from build123d import *

# Parameters (mm, degrees)
BOSS_EXTRUDE1_DEPTH      = 600
SKETCH2_R                = 15
BOSS_EXTRUDE2_DEPTH      = 30
BOSS_EXTRUDE3_DEPTH      = 12
BOSS_EXTRUDE3_DEPTH_BACK = 12
SKETCH3_R                = 15
SKETCH4_W                = 64.999273694
SKETCH4_H                = 54.968001075
CUT_EXTRUDE1_DEPTH       = 5
CUT_EXTRUDE2_DEPTH       = 621.826062597


with BuildPart() as part:
    # Sketch1 → Boss-Extrude1 (new body)
    with BuildSketch(Plane(origin=(0, 0, 0), x_dir=(1, 0, 0), z_dir=(0, 1, 0))):
        Polygon((-20, 40), (-20, 60), (50, 60), (50, -60), (-20, -60), (-20, -40), (20, -40), (20, 40), align=None)
    extrude(amount=BOSS_EXTRUDE1_DEPTH)

    # Sketch2 → Boss-Extrude2 (add)
    with BuildSketch(Plane(origin=(0, 0, -60), x_dir=(-1, 0, 0), z_dir=(0, 0, -1))):
        with BuildLine():
            Line((-34.984231122, 36.653571932), (-80, 36.653571932))
            ThreePointArc((-80, 36.653571932), (-105, 61.653571932), (-80, 86.653571932))
            Line((-80, 86.653571932), (-34.984231122, 86.653571932))
            Line((-34.984231122, 86.653571932), (-34.984231122, 36.653571932))
        make_face()
        with Locations((-80, 61.653571932)):
            Circle(SKETCH2_R, mode=Mode.SUBTRACT)
    boss_extrude2 = extrude(amount=-BOSS_EXTRUDE2_DEPTH)

    # Mirror1: Boss-Extrude2 across plane
    add(boss_extrude2.mirror(Plane.XY))

    # Sketch3 → Boss-Extrude3 (add, two sides: drawn at the far end of the back side and taken through both)
    with BuildSketch(Plane.XY.offset(-BOSS_EXTRUDE3_DEPTH_BACK)):
        with BuildLine():
            Line((42.373646318, 600), (75, 600))
            ThreePointArc((75, 600), (100, 575), (75, 550))
            Line((75, 550), (42.373646318, 550))
            Line((42.373646318, 550), (42.373646318, 600))
        make_face()
        with Locations((75, 575)):
            Circle(SKETCH3_R, mode=Mode.SUBTRACT)
    extrude(amount=BOSS_EXTRUDE3_DEPTH + BOSS_EXTRUDE3_DEPTH_BACK)

    # Sketch4 → Cut-Extrude1 (cut)
    with BuildSketch(Plane(origin=(0, 0, -60), x_dir=(-1, 0, 0), z_dir=(0, 0, -1))):
        with Locations((-82.499636847, 64.13757247)):
            Rectangle(SKETCH4_W, SKETCH4_H)
    cut_extrude1 = extrude(amount=-CUT_EXTRUDE1_DEPTH, mode=Mode.SUBTRACT)

    # Mirror2: Cut-Extrude1 across plane
    add(cut_extrude1.mirror(Plane.XY), mode=Mode.SUBTRACT)

    # Sketch5 → Cut-Extrude2 (cut, through all)
    with BuildSketch(Plane(origin=(0, 0, -60), x_dir=(-1, 0, 0), z_dir=(0, 0, -1))):
        Polygon((-50, 30.340627067), (-30, 0), (-50, 0), align=None)
    extrude(amount=-CUT_EXTRUDE2_DEPTH, mode=Mode.SUBTRACT)


solid = part.part
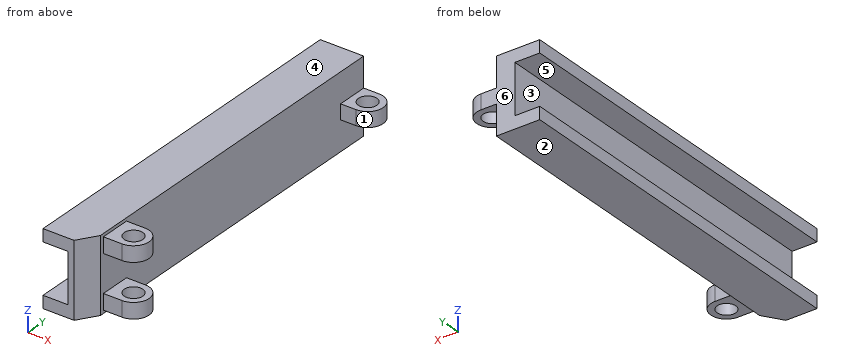
Input: part model. Units: mm. Frame: model coordinates. Face numbers are marked on the shaded views. A direction names the side the tool comes from. Give positions to 0.01 mm unless a question says otherwise; leave off trailing zeros. Loops run counter-clockwise (first coordinate to the right, second up) from the corner with the lowest first, then second, coordinate; pieces in that order, holes last. Notation, with made-up numbers: M 41,53.5 L 47,53.5 A16 cw 47,62.5 Z; hole C -11,60 d5. An arc over 180 degrees is marked long. Use CSV: the item, a comma, the result in double quotes.
(1) Section A-A, the plane y = 575. Return loops of the section in (x, z).
Outcome:
outline,"M -20,-60 L 50,-60 L 50,-12 L 60,-12 L 60,12 L 50,12 L 50,60 L -20,60 L -20,40 L 20,40 L 20,-40 L -20,-40 Z; M 90,-12 L 100,-12 L 100,12 L 90,12 Z"
(2) Section C-C, the plane y = 102.5. Return loops of the section in (x, z), plus the area to 3 significant figures.
Outcome:
outline,"M -20,-60 L 50,-60 L 50,60 L -20,60 L -20,40 L 20,40 L 20,-40 L -20,-40 Z"
area,"5,200 mm²"
(3) Set-up query: the marked faces 5 and 6. Return all of +Z, -Z, +X, -X, +Y, -Y with unobstructed straight access to the full face (end or side cutting, diameter ignored); none if empty.
Outcome:
face 5,"-X, +Y, -Y"
face 6,"+Z, -Z, +X, -X, +Y"
(4) Material intervals for L1, parallel to Y at x = 80, z = -41; L2, parallel to Z at x = -9, y = 549; L3, parallel to X at y = 575, z = 3, sorted ascending. Write a range as [from, to].
Outcome:
L1,"y = [36.65, 46.65], [76.65, 86.65]"
L2,"z = [-60, -40], [40, 60]"
L3,"x = [20, 60], [90, 100]"
(5) Pull-direction query (Z, two-part tool) for the marked faces 1, 2, 3 and 4; classes: pulls with the +Z half, pulls with the -Z half, needs draft (parallel to the pull), parting line crosses it, or undercut.
Outcome:
face 1,"needs draft"
face 2,"pulls with the -Z half"
face 3,"undercut"
face 4,"pulls with the +Z half"
(6) Section B-B, the plane z = -19. Return loops of the section in (x, y).
Outcome:
outline,"M 20,0 L 30,0 L 50,30.34 L 50,600 L 20,600 Z"
(7) Pin query (flat end, axial travel): P1, Ø1, axis at x = 51.5, y = 131.5, coming from the +Z side; P2, Ø3, axis at y = 517.5, z = -24.5, coming from the -X side; P3, Ø7.5, axis at x = 66, z = 39, coming from the -Y side; P4, Ø10, axis at y = 392.5, z = 32.5, coming from the +X side. Return the tip coordinate at first contact, or that it passes through.
Outcome:
P1,"passes through"
P2,"stops at x = 20"
P3,"stops at y = 36.65"
P4,"stops at x = 50"
